Part print with two shaded views. Sizes in mm from the minimum x, y, z corner. Round coordinates to 2 decimals unless told otherwise and drop trailing zeros. Loops run counter-clockwise (first coordinate to the right, second up) from the corner with the lowest first, then second, coordinate; pieces in that order, holes last. Notation, with made-up numbers: M 87,-24 L 95,-24 A29 cw 95,13 Z; hole C 35.5,58 d6. An arc over 180 degrees is marked long. Put each result on its own line as item: value. Start each with the question number.
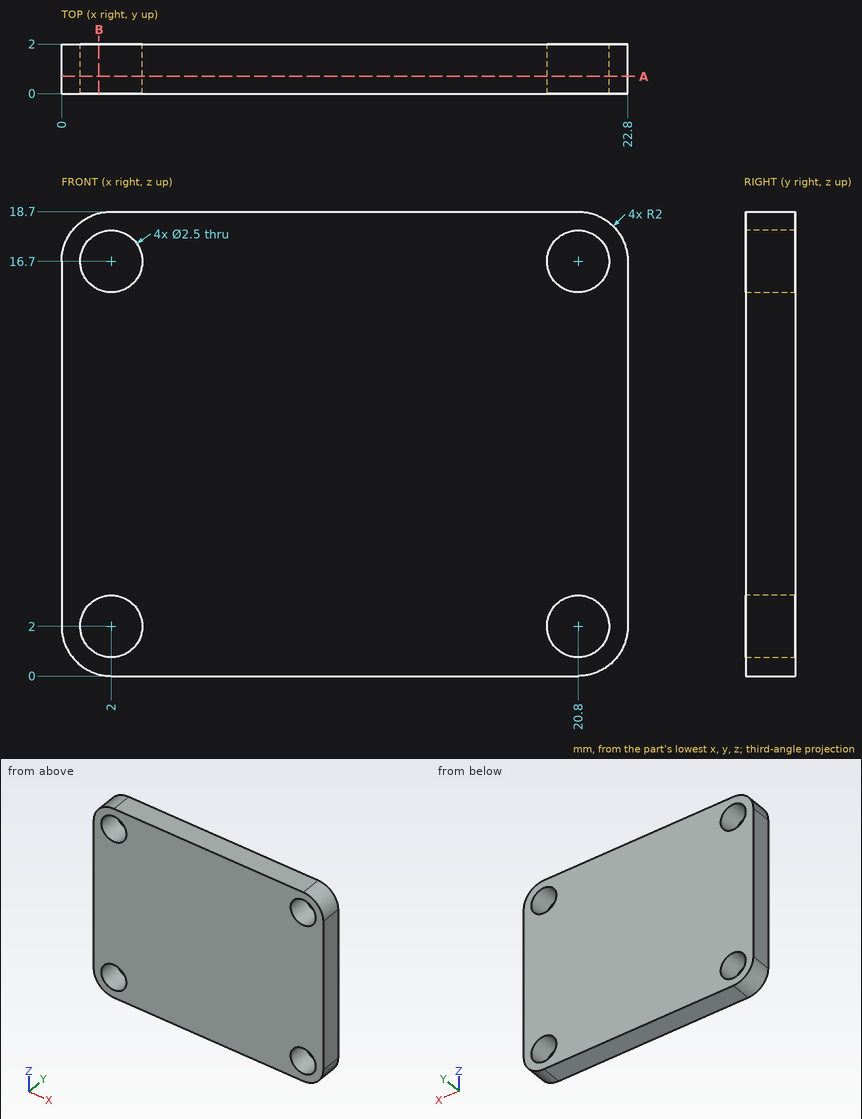
(1) Cut at B-B on x = 1.5. List the corners of the cut face in (y, z), and give its area (3 significant figures).
(2) Cut at A-A on y = 0.7. List the corners of the cut face in (x, z).
(3) Drill centre lines: line 1 along X through (y, z) = (1.2, 2); line 2 along Z through (x, y) = (20.75, 0.3); line 3 along X through (y, z) = (1.85, 15.75). Where is each one in solid material? Low to high.
Taken from the geometry:
1. outline: M 0,0.06 L 2,0.06 L 2,0.85 L 0,0.85 Z; M 0,3.15 L 2,3.15 L 2,15.55 L 0,15.55 Z; M 0,17.85 L 2,17.85 L 2,18.64 L 0,18.64 Z
1. area: 28.0 mm2
2. outline: M 0,2 A2 ccw 2,0 L 20.8,0 A2 ccw 22.8,2 L 22.8,16.7 A2 ccw 20.8,18.7 L 2,18.7 A2 ccw 0,16.7 Z; hole C 2,2 d2.5; hole C 2,16.7 d2.5; hole C 20.8,2 d2.5; hole C 20.8,16.7 d2.5
3. line 1: 0 to 0.75, 3.25 to 19.55, 22.05 to 22.8
3. line 2: 0 to 0.75, 3.25 to 15.45, 17.95 to 18.7
3. line 3: 0 to 1.19, 2.81 to 19.99, 21.61 to 22.8
